```python
from build123d import *


with BuildPart() as part:
    # Sketch1 → Revolve1 (revolve)
    with BuildSketch(Plane.XY):
        Polygon((-70, 70), (-70, 71.5), (-66, 72.65), (-66, 75), (-61.7, 75), (-61.7, 70), (-64.127855471, 70), (-64.127855471, 70.546927726), (-65.050124916, 70), align=None)
    revolve(axis=Axis((0, 0, 0), (-1, 0, 0)))


solid = part.part
```
Read the model definition and answer for the solid it produces. Units are mm, in the model's axes. Round coordinates to 2 decimals unless told otherwise and drop trailing zeros. Write each loop counter-clockwise with the first axis right and the second up, starting at its lowest first coordinate (ties: lowest second). Pieces come first, ordered by that corner, then holes. Notation, with made-up numbers: (36, 28.25) -> (43, 28.25) arc R23 ccw to (43, 39.25) -> close; hole circle Ø10 at (22, -22.5). An arc over 180 degrees is marked (long way). Answer in a Markdown table with one row per item. Add a question column.
1) Given P1, Ø4, axis at x = -69, y = -6.5, coming from the -Z side; P2, Ø3, axis at x = -66.5, z = -1, coming from the +Y side, each flat-ended and moving along its own axis, determine where each tip first touches the part or whether it passes through.
2) Find section C-C, the plane x = -68.25. Determine the outline of the cut face in (y, z).
3) Consider line 1 (Z direction, x = -62.6, y = 0); line 2 (Z direction, x = -66.1, y = 0). Determine where each line is inside the solid, lowest interval first.
4) Determine the mould class of faces 1 (the face through (-66, 39.2, -61.5)), 2 (the face through (-63.82, -9.764, -74.362)), 3 (the face through (-67.56, -55.55, 42.594)), 4 (the face through (-62.931, -55.55, 42.594)) for opening direction Y: pulls with the +Y half, pulls with the -Y half, needs draft (parallel to the pull), parting line crosses it, or undercut.
5) Find section A-A, the plane z = 0. Determine the outline of the cut face in (x, y).
Findings below:
| question | item | result |
|---|---|---|
| 1 | P1 | z = -72.1 |
| 1 | P2 | y = 75 |
| 2 | outline | circle Ø144.01 at (0, 0); hole circle Ø140 at (0, 0) |
| 3 | line 1 | -75 to -70, 70 to 75 |
| 3 | line 2 | -72.62 to -70, 70 to 72.62 |
| 4 | face 1 | needs draft |
| 4 | face 2 | parting line crosses it |
| 4 | face 3 | undercut |
| 4 | face 4 | undercut |
| 5 | outline | (-70, -71.5) -> (-66, -72.65) -> (-66, -75) -> (-61.7, -75) -> (-61.7, -70) -> (-64.13, -70) -> (-64.13, -70.55) -> (-65.05, -70) -> (-70, -70) -> close; (-70, 70) -> (-65.05, 70) -> (-64.13, 70.55) -> (-64.13, 70) -> (-61.7, 70) -> (-61.7, 75) -> (-66, 75) -> (-66, 72.65) -> (-70, 71.5) -> close |
